The listing builds one solid part. Answer for the finished solid, in the listing's coordinates (mm). A direction names the side the tool comes from. Give positions to 0.01 mm unless a question says otherwise; leave off trailing zeros. Order: outer loops, then holes, each group sorted by start corner. A loop starts at its lowest first (then second) coordinate and runs counter-clockwise, first axis right, second up.
```python
from build123d import *

# Parameters (mm, degrees)
SKETCH1_R           = 1.5
BOSS_EXTRUDE1_DEPTH = 6.2
SKETCH3_R           = 0.2
CUT_EXTRUDE2_DEPTH  = 7.55286197
CHAMFER1_SIZE       = 3
CHAMFER1_SIZE2      = 1
SKETCH5_R           = 0.5
CUT_EXTRUDE3_DEPTH  = 1.5
BOSS_EXTRUDE2_START = 1.5
SKETCH7_R           = 0.5
BOSS_EXTRUDE2_DEPTH = 1.5
BOSS_EXTRUDE3_START = 3
SKETCH8_R           = 2
SKETCH8_R_2         = 0.5
BOSS_EXTRUDE3_DEPTH = 3
CHAMFER4_SIZE       = 0.2


with BuildPart() as part:
    # Sketch1 → Boss-Extrude1 (new body)
    with BuildSketch(Plane(origin=(0, 0, 0), x_dir=(1, 0, 0), z_dir=(0, 1, 0))):
        with Locations(Location((0, 0, 0), (0, 0, 90))):
            Circle(SKETCH1_R)
    extrude(amount=BOSS_EXTRUDE1_DEPTH)

    # Sketch3 → Cut-Extrude2 (cut, through all)
    with BuildSketch(Plane(origin=(0, 6.2, 0), x_dir=(1, 0, 0), z_dir=(0, 1, 0))):
        with Locations(Location((0, 0, 0), (0, 0, 270))):
            Circle(SKETCH3_R)
    extrude(amount=-CUT_EXTRUDE2_DEPTH, mode=Mode.SUBTRACT)

    # Chamfer1
    chamfer1_edges = [part.edges().sort_by_distance(p)[0] for p in [
        (0, 6.2, 1.5),
    ]]
    chamfer1_side = [part.faces().sort_by_distance(p)[0] for p in [
        (0, 3.1, 1.5),
    ]]
    chamfer(chamfer1_edges, length=CHAMFER1_SIZE, length2=CHAMFER1_SIZE2, reference=chamfer1_side[0])

    # Sketch5 → Cut-Extrude3 (cut)
    with BuildSketch(Plane.XZ):
        with Locations(Location((0, 0, 0), (0, 0, 270))):
            Circle(SKETCH5_R)
    extrude(amount=-CUT_EXTRUDE3_DEPTH, mode=Mode.SUBTRACT)

    # Sketch7 → Boss-Extrude2 (add)
    with BuildSketch(Plane.XZ.offset(BOSS_EXTRUDE2_START)):
        Polygon((0, 2.598076211), (-2.25, 1.299038106), (-2.25, -1.299038106), (0, -2.598076211), (2.25, -1.299038106), (2.25, 1.299038106), align=None)
        with Locations(Location((0, 0, 0), (0, 0, 270))):
            Circle(SKETCH7_R, mode=Mode.SUBTRACT)
    extrude(amount=-BOSS_EXTRUDE2_DEPTH)

    # Sketch8 → Boss-Extrude3 (add)
    with BuildSketch(Plane.XZ.offset(1.5).offset(BOSS_EXTRUDE3_START)):
        with Locations(Location((0, 0, 0), (0, 0, 270))):
            Circle(SKETCH8_R)
        with Locations(Location((0, 0, 0), (0, 0, 270))):
            Circle(SKETCH8_R_2, mode=Mode.SUBTRACT)
    extrude(amount=-BOSS_EXTRUDE3_DEPTH)

    # Sketch9 → Cut-Revolve2 (revolve, cut)
    with BuildSketch(Plane.XY, mode=Mode.PRIVATE) as cut_revolve2_sk:
        Polygon((0.2, 6.2), (1.1, -4.5), (0, -4.5), (0, 6.2), align=None)
    revolve(cut_revolve2_sk.sketch.rotate(Axis((0, -1009.643261514, 0), (0, 1, 0)), 90), axis=Axis((0, -1009.643261514, 0), (0, 1, 0)), mode=Mode.SUBTRACT)

    # Chamfer4
    chamfer4_edges = [part.edges().sort_by_distance(p)[0] for p in [
        (0, -4.5, 2),
    ]]
    chamfer(chamfer4_edges, length=CHAMFER4_SIZE)


solid = part.part
```
1) A tool of negligible diameter and unlimited length cuts with its end or side. For faces 1 (the flat face through (-2, 0, 0)), 2 (the cylindrical face through (-2, -3, 0)), 3 (the flat face through (-1.109, -0.76, 1.958)), from which of +Z, -Z, +X, -X, +Y, -Y can it reach the whole face along a straight path? Write none if from no direction.
Geometry says:
face 1: +Y
face 2: -Y
face 3: +Z, -X, +Y, -Y
2) Find section D-D (y = 3.75). Write down the section's boundary in (x, z).
Geometry says:
outline: circle Ø2.63 at (0, 0); hole circle Ø0.81 at (0, 0)
3) Find section B-B (y = -0.25). Write down the section's boundary in (x, z).
Geometry says:
outline: (-2.25, -1.3) - (0, -2.6) - (2.25, -1.3) - (2.25, 1.3) - (0, 2.6) - (-2.25, 1.3) - close; hole circle Ø1.49 at (0, 0)
4) Straight lines are drawn through the part: probe 1 along X at (y, z) = (-3, -0.45); probe 2 along Y at (x, z) = (-1.7, 1.45); probe 3 along Z at (x, y) = (-0.15, 0.5). For each, find the intervals that lie inside material, in ascending order.
Geometry says:
probe 1: x = -1.95 to -0.86, 0.86 to 1.95
probe 2: y = -1.5 to 0
probe 3: z = -1.49 to -0.66, 0.66 to 1.49
5) Find section C-C (y = 1). Write down the section's boundary in (x, z).
Geometry says:
outline: circle Ø3 at (0, 0); hole circle Ø1.27 at (0, 0)
6) For a pull along X with two mould halves and no side action, classify faces 4 (the flat face through (-1, -4.5, 1)), 5 (the conical face through (0.4, 0.78, 0.52)), 6 (the flat face through (1.14, -0.76, 1.94)) as +X half, -X half, draft (parallel to the pull), parting line (faces both ways), or undercut.
Geometry says:
face 4: draft
face 5: undercut
face 6: +X half
7) Find section A-A (z = 0). Write down the section's boundary in (x, y), then the cut area to 3 significant figures.
Geometry says:
outline: (-2.25, -1.5) - (-2, -1.5) - (-2, -4.3) - (-1.8, -4.5) - (-1.1, -4.5) - (-0.2, 6.2) - (-0.5, 6.2) - (-1.5, 3.2) - (-1.5, 0) - (-2.25, 0) - close; (0.2, 6.2) - (1.1, -4.5) - (1.8, -4.5) - (2, -4.3) - (2, -1.5) - (2.25, -1.5) - (2.25, 0) - (1.5, 0) - (1.5, 3.2) - (0.5, 6.2) - close
area: 20.4 mm2
8) Given P1, Ø1, axis at x = -1, y = 1.5, coming from the -Z side, flat-ended and moving along its own axis, determine where the tip first touches the part or whether it passes through.
Geometry says:
P1: stops at z = -1.41
